CAD build for the part. Positions are in the model's coordinates, mm. Face numbers are marked on the shaded views. Coordinates: 2 decimals unless noted, no trailing zeros. Loops run counter-clockwise (first coordinate to the right, second up) from the corner with the lowest first, then second, coordinate; pieces in that order, holes last. Notation, with made-up numbers: (-19, 28.25) -> (5, 28.25) arc R21 ccw to (5, 38.25) -> close; hole circle Ø10 at (-3, 23). An arc over 180 degrees is marked (long way). Return JSON: item names as keys, results as strings. Group by question number.
(1) Saw through at C-C on z = -84. Write the cut outline in (x, y), then the cut area to 3 significant figures.
(2) Mould opens along Z. For the marked faces 1 and 2 say: pulls with the +Z half, pulls with the -Z half, needs draft (parallel to the pull), parting line crosses it, or undercut.
(3) Probe L1, parallel to X at y = 143.25, z = 0; L2, parallel to Y at x = -32.5, z = 60.5; L3, parallel to Z at x = 23, y = 152.75. List the from-to ranges inside material, lowest first.
(4) Saw through at B-B on z = 0. Write the cut outline in (x, y), then the cut area to 3 significant figures.
(5) Saw through at A-A on x = 0. Write the cut outline in (y, z).
(6) Saw through at D-D on x = 68. Write the cut outline in (y, z).
(7) Flat gauge pins, fed straight in: pin 1 Ø2 at (x, y) = (2, 144.5) entering from -Z; pin 2 Ø12 at (x, y) = (60.5, 146.5) entering from +Z; pin 3 Ø8 at (x, y) = (-51.5, 148.5) entering from -Z. Where does each tip first touch, or does it go through?
```python
from build123d import *


with BuildPart() as part:
    # Sketch1 → Revolve1 (revolve)
    with BuildSketch(Plane.XY, mode=Mode.PRIVATE) as revolve1_sk:
        Polygon((102, 158), (65.583048881, 158), (65.583048881, 151.5), (63.995706961, 151.5), (63.995706961, 137.5), (60.995706961, 137.5), (60.995706961, 153.778962031), (63.193534924, 153.778962031), (63.193534924, 160.531936258), (102, 160.531936258), align=None)
    revolve(revolve1_sk.sketch.rotate(Axis((0, 0, 0), (0, -1, 0)), 90), axis=Axis((0, 0, 0), (0, -1, 0)))


solid = part.part
```
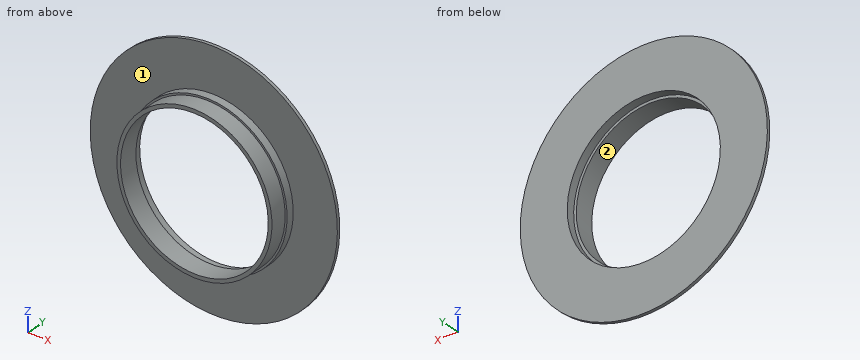
Geometry results:
{
 "1": {"outline": "(-57.86, 158) -> (57.86, 158) -> (57.86, 160.53) -> (-57.86, 160.53) -> close", "area": "293 mm²"},
 "2": {"face 1": "needs draft", "face 2": "undercut"},
 "3": {"L1": "-64 to -61, 61 to 64", "L2": "158 to 160.53", "L3": "-61.42 to -56.49, 56.49 to 61.42"},
 "4": {"outline": "(-102, 158) -> (-65.58, 158) -> (-65.58, 151.5) -> (-64, 151.5) -> (-64, 137.5) -> (-61, 137.5) -> (-61, 153.78) -> (-63.19, 153.78) -> (-63.19, 160.53) -> (-102, 160.53) -> close; (61, 137.5) -> (64, 137.5) -> (64, 151.5) -> (65.58, 151.5) -> (65.58, 158) -> (102, 158) -> (102, 160.53) -> (63.19, 160.53) -> (63.19, 153.78) -> (61, 153.78) -> close", "area": "322 mm²"},
 "5": {"outline": "(137.5, -64) -> (151.5, -64) -> (151.5, -65.58) -> (158, -65.58) -> (158, -102) -> (160.53, -102) -> (160.53, -63.19) -> (153.78, -63.19) -> (153.78, -61) -> (137.5, -61) -> close; (137.5, 61) -> (153.78, 61) -> (153.78, 63.19) -> (160.53, 63.19) -> (160.53, 102) -> (158, 102) -> (158, 65.58) -> (151.5, 65.58) -> (151.5, 64) -> (137.5, 64) -> close"},
 "6": {"outline": "(158, -76.03) -> (160.53, -76.03) -> (160.53, 76.03) -> (158, 76.03) -> close"},
 "7": {"pin 1": "z = -63.99", "pin 2": "z = 33.54", "pin 3": "z = -43.75"}
}
